from build123d import *

# Parameters (mm, degrees)
EXTRUDE_THIN1_DEPTH = 100


with BuildPart() as part:
    # Sketch1 → Extrude-Thin1 (new body)
    with BuildSketch(Plane.XY):
        with BuildLine():
            Line((0, -130), (0, -50))
            ThreePointArc((0, -50), (14.644660941, -14.644660941), (50, 0))
            Line((50, 0), (130, 0))
            Line((130, 0), (130, -16))
            Line((130, -16), (50, -16))
            ThreePointArc((50, -16), (25.95836944, -25.95836944), (16, -50))
            Line((16, -50), (16, -130))
            Line((16, -130), (0, -130))
        make_face()
    extrude(amount=EXTRUDE_THIN1_DEPTH)


solid = part.part
Could you check a few things on this model? Use its own coordinates, in mm. A direction names the side the tool comes from. Coordinates: 2 decimals unless noted, no trailing zeros. Write each loop counter-clockwise with the first axis right and the second up, starting at its lowest first coordinate (ties: lowest second). Pieces come first, ordered by that corner, then holes. Notation, with made-up numbers: (4.25, 58.25) - (31.25, 58.25) arc R19 cw to (31.25, 77.25) - close; hole circle Ø8 at (81.5, -22). An arc over 180 degrees is marked (long way). Write item = value, one per line.
1) For faces 1 (the flat face through (130, -8, 49)), 2 (the flat face through (16, -89, 49)), which set-ups out of +Z, -Z, +X, -X, +Y, -Y let a thin tool reach every point of the face, with its end or its side?
Result set:
face_1 = +Z, -Z, +X, +Y, -Y
face_2 = +Z, -Z, +X, -Y
2) Suppose I cut it at B-B on x = 96. Please give me the cut outline in (y, z), plus the area to 3 significant figures.
Result set:
outline = (-16, 0) - (0, 0) - (0, 100) - (-16, 100) - close
area = 1,600 mm2
3) Suppose I cut it at C-C on y = -83.5. Please give me the cut outline in (x, z), plus the area to 3 significant figures.
Result set:
outline = (0, 0) - (16, 0) - (16, 100) - (0, 100) - close
area = 1,600 mm2
4) Please list where these lines run through material, in increasing order: line 1 (Y direction, x = 92.5, z = 49); line 2 (X direction, y = -57, z = 15.5); line 3 (Y direction, x = 41, z = 51). Write a range as [from, to].
Result set:
line_1 = [-16, 0]
line_2 = [0, 16]
line_3 = [-17.21, -0.82]
5) Will this pin go through, and if not, where does the flat tip stop? pin 1 Ø4 at (x, z) = (50.5, 15) entering from -Y.
Result set:
pin_1 = -16.03
6) Suppose I cut it at A-A on z = 63. Please give me the cut outline in (x, y).
Result set:
outline = (0, -130) - (16, -130) - (16, -50) arc R34 cw to (50, -16) - (130, -16) - (130, 0) - (50, 0) arc R50 ccw to (0, -50) - close
